The listing builds one solid part. Answer for the finished solid, in the listing's coordinates (mm). A direction names the side the tool comes from. Coordinates: 2 decimals unless noted, no trailing zeros. Write each loop counter-clockwise with the first axis right and the second up, starting at its lowest first coordinate (ties: lowest second). Pieces come first, ordered by that corner, then holes. Notation, with made-up numbers: M -35,51.25 L -10,51.25 A9 cw -10,66.25 Z; hole C -23.75,-39.5 d11. An arc over 180 degrees is marked long. Write item = value, one per line. Start each with the question number.
```python
from build123d import *

# Parameters (mm, degrees)
SKETCH1_W                = 60
SKETCH1_H                = 150
BOSS_EXTRUDE1_DEPTH      = 10
SKETCH2_R                = 5
CUT_EXTRUDE1_DEPTH       = 10
BOSS_EXTRUDE2_DEPTH      = 20
BOSS_EXTRUDE2_DEPTH_BACK = 80.0001
SKETCH3_R                = 5
BOSS_EXTRUDE3_DEPTH      = 5
BOSS_EXTRUDE3_DEPTH_BACK = 105
SKETCH4_R                = 2.5


with BuildPart() as part:
    # Sketch1 → Boss-Extrude1 (new body)
    with BuildSketch(Plane.XY):
        Rectangle(SKETCH1_W, SKETCH1_H)
    extrude(amount=BOSS_EXTRUDE1_DEPTH)

    # Sketch2 → Cut-Extrude1 (cut)
    with BuildSketch(Plane.XY.offset(10)):
        with Locations((-16.71752283, 0)):
            Circle(SKETCH2_R)
        with Locations((19.976362571, 0)):
            Circle(SKETCH2_R)
    extrude(amount=-CUT_EXTRUDE1_DEPTH, mode=Mode.SUBTRACT)

    # Sketch3 → Boss-Extrude2 (add, two sides: drawn at the far end of the back side and taken through both)
    with BuildSketch(Plane(origin=(30, 0, 0), x_dir=(0, 0, -1), z_dir=(1, 0, 0)).offset(-BOSS_EXTRUDE2_DEPTH_BACK)):
        with Locations((-5, 75)):
            Circle(SKETCH3_R)
    extrude(amount=BOSS_EXTRUDE2_DEPTH + BOSS_EXTRUDE2_DEPTH_BACK)

    # Sketch4 → Boss-Extrude3 (add, two sides: drawn at the far end of the back side and taken through both)
    with BuildSketch(Plane.ZY.offset(50.0001).offset(-BOSS_EXTRUDE3_DEPTH_BACK)):
        with Locations((5, 75)):
            Circle(SKETCH4_R)
    extrude(amount=BOSS_EXTRUDE3_DEPTH + BOSS_EXTRUDE3_DEPTH_BACK)


solid = part.part
```
1. The part is cut by section A-A, the plane y = 0. Write down the section's boundary in (x, z).
2. The part is cut by section D-D, the plane y = 27.5. Write down the section's boundary in (x, z).
3. For a pull along Y with two mould halves and no side action, classify faces 5 (the face through (-55, 75, 5)), 6 (the face through (14.98, 0.22, 5.07)), 7 (the face through (0, -75, 5)) as pulls with the +Y half, pulls with the -Y half, needs draft (parallel to the pull), parting line crosses it, or undercut.
4. The part is cut by section C-C, the plane x = 47. Write down the section's boundary in (y, z).
5. Each of these flat-tipped pins is pushed along its axis until it touches: pin 1 (5 mm diameter, centred on y = 35, z = 4, fed in from -X); pin 2 (6 mm diameter, centred on x = 19.98, y = 0, fed in from +Z). Where does it stop, or does it pass through?
6. For faces 1 (the face through (50, 73, 3)), 2 (the face through (-50, 73, 3)), 3 (the face through (-0.7, 79.957, 5.651)), 4 (the face through (55, 75, 5)), determine the directions among +Z, -Z, +X, -X, +Y, -Y from which every point of the face is accessible in a straight line to the end or side of a thin tool.
7. Straight lines are drawn through the part: L1, parallel to X at y = 4.5, z = 8.25; L2, parallel to X at y = 35, z = 6.5; L3, parallel to Y at x = 17.5, z = 5.25. For each, find the intervals that lie inside material, in ascending order. Write a range as [from, to].
8. The part is cut by section B-B, the plane z = 5. Write down the section's boundary in (x, y).
Solution:
q1.outline = M -30,0 L -21.72,0 L -21.72,10 L -30,10 Z; M -11.72,0 L 14.98,0 L 14.98,10 L -11.72,10 Z; M 24.98,0 L 30,0 L 30,10 L 24.98,10 Z
q2.outline = M -30,0 L 30,0 L 30,10 L -30,10 Z
q3.face_5 = needs draft
q3.face_6 = undercut
q3.face_7 = pulls with the -Y half
q4.outline = C 75,5 d10
q5.pin_1 = -30
q5.pin_2 = through
q6.face_1 = +X
q6.face_2 = -X
q6.face_3 = none
q6.face_4 = +Z, -Z, +X, +Y, -Y
q7.L1 = [-30, -18.9], [-14.54, 17.8], [22.16, 30]
q7.L2 = [-30, 30]
q7.L3 = [-75, -4.34], [4.34, 79.99]
q8.outline = M -55,72.5 L -50,72.5 L -50,70 L -30,70 L -30,-75 L 30,-75 L 30,70 L 50,70 L 50,72.5 L 55,72.5 L 55,77.5 L 50,77.5 L 50,80 L -50,80 L -50,77.5 L -55,77.5 Z; hole C -16.72,0 d10; hole C 19.98,0 d10
